Geometry check sheet. Reference: the model listing, model coordinates, mm. Give positions to 0.01 mm unless a question says otherwise; leave off trailing zeros. Loops run counter-clockwise (first coordinate to the right, second up) from the corner with the lowest first, then second, coordinate; pieces in that order, holes last.
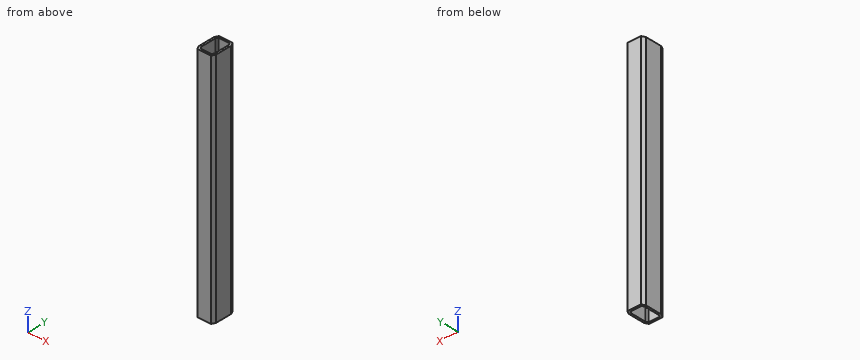
```python
from build123d import *

# Parameters (mm, degrees)
BOSS_EXTRUDE1_DEPTH = 600


with BuildPart() as part:
    # Sketch1 → Boss-Extrude1 (new body)
    with BuildSketch(Plane.XY):
        Polygon((-17.319660113, 136.5), (17.319660113, 136.5), (22, 127.139320225), (22, 85.160679775), (17.319660113, 75.8), (-17.319660113, 75.8), (-22, 85.160679775), (-22, 127.139320225), align=None)
        Polygon((-14.229490169, 131.5), (14.229490169, 131.5), (17, 125.958980338), (17, 86.341019662), (14.229490169, 80.8), (-14.229490169, 80.8), (-17, 86.341019662), (-17, 125.958980338), align=None, mode=Mode.SUBTRACT)
    extrude(amount=BOSS_EXTRUDE1_DEPTH)


solid = part.part
```
1) Scan lines: line 1 along X through (y, z) = (97, 295.5); line 2 along Y through (x, z) = (-1, 100); line 3 along Y through (x, z) = (-16, 176). Record each from-to range of solid material in increasing order.
2) Sectioned sample at C-C on z = 276. Enter the section's corners in (x, y), plus the area to 3 significant figures.
3) Sectioned sample at B-B on x = -0.5. Enter the section's corners in (y, z), plus the area to 3 significant figures.
4) Sectioned sample at A-A on y = 102.5. Enter the section's corners in (x, z).
Determined:
1. line 1: x = -22 to -17, 17 to 22
1. line 2: y = 75.8 to 80.8, 131.5 to 136.5
1. line 3: y = 75.8 to 84.34, 127.96 to 136.5
2. outline: (-22, 85.16) - (-17.32, 75.8) - (17.32, 75.8) - (22, 85.16) - (22, 127.14) - (17.32, 136.5) - (-17.32, 136.5) - (-22, 127.14) - close; hole (-17, 86.34) - (-14.23, 80.8) - (14.23, 80.8) - (17, 86.34) - (17, 125.96) - (14.23, 131.5) - (-14.23, 131.5) - (-17, 125.96) - close
2. area: 890 mm2
3. outline: (75.8, 0) - (80.8, 0) - (80.8, 600) - (75.8, 600) - close; (131.5, 0) - (136.5, 0) - (136.5, 600) - (131.5, 600) - close
3. area: 6,000 mm2
4. outline: (-22, 0) - (-17, 0) - (-17, 600) - (-22, 600) - close; (17, 0) - (22, 0) - (22, 600) - (17, 600) - close
